Job drawing, mm, ordinate dimensions from the low corner. One solid piece. A direction names the side the tool comes from. Give positions to 0.01 mm unless a question says otherwise; leave off trailing zeros. Loops run counter-clockwise (first coordinate to the right, second up) from the corner with the lowest first, then second, coordinate; pieces in that order, holes last. Notation, with made-up numbers: (31, -6) - (80, -6) arc R31 ccw to (80, 33) - close; hole circle Ø3 at (-19, 24). An arc over 180 degrees is marked (long way). Answer as CSV lines item,"result". Start each with the question number.
Item 1: Pull direction Z, two halves, no side cores. Call the marked faces 1, 2 and 3: pulls with the +Z half, pulls with the -Z half, needs draft (parallel to the pull), parting line crosses it, or undercut.
Item 2: Saw through at B-B on y = 6.5. Give the cut face in (x, z).
Item 3: Saw through at D-D on z = 29.5. Give the cut face in (x, y), plus the area to 3 significant figures.
Item 4: Drill centre lines: L1, parallel to Z at x = 60, y = 3.9; L2, parallel to X at y = 4, z = 50; L3, parallel to Z at x = 23, y = 5.5. Where is each one in solid material? Low to high. Write a range as from..to.
Item 5: Saw through at A-A on x = 60. Give the cut face in (y, z), plus the area to 3 significant figures.
Item 6: Saw through at C-C on z = 15. Give the cut face in (x, y).
Item 7: Tool access for the marked faces 4, 5 and 6: list every direction of +Z, -Z, +X, -X, +Y, -Y with a clear straight run to the whole face (end or side of a thin tool).
Item 8: Pin check, flat tips, straight feed: pin 1 (19.5 mm diameter, centred on x = 43.5, z = 41, fed in from +Y); pin 2 (8 mm diameter, centred on x = 60, z = 15, fed in from -Y); pin 3 (3 mm diameter, centred on y = 26, z = 46, fed in from +X). Stop position of each tip, or through.
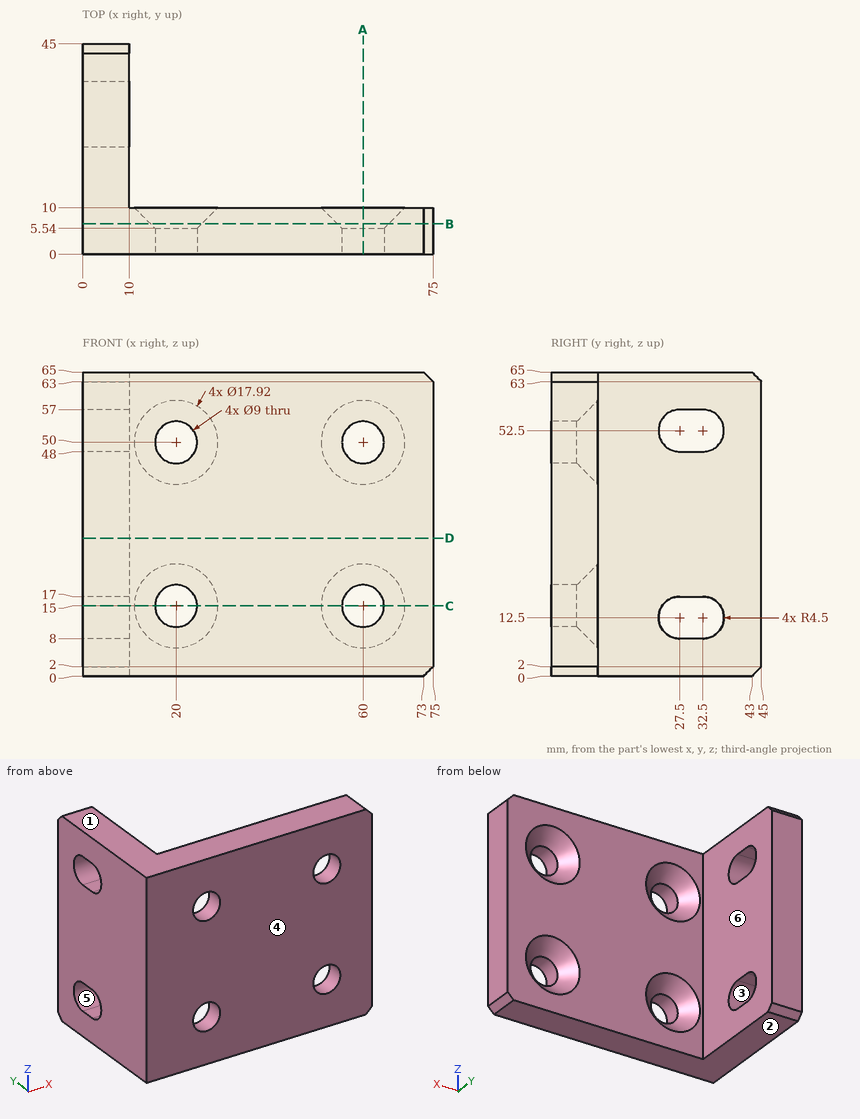
Responses:
1,face 1,"pulls with the +Z half"
1,face 2,"pulls with the -Z half"
1,face 3,"undercut"
2,outline,"(0, 0) - (73, 0) - (75, 2) - (75, 63) - (73, 65) - (0, 65) - close; hole circle Ø10.92 at (20, 15); hole circle Ø10.92 at (20, 50); hole circle Ø10.92 at (60, 15); hole circle Ø10.92 at (60, 50)"
3,outline,"(0, 0) - (75, 0) - (75, 10) - (10, 10) - (10, 45) - (0, 45) - close"
3,area,"1,100 mm2"
4,L1,"0..10.5, 19.5..45.5, 54.5..65"
4,L2,"0..15.5, 24.5..55.5, 64.5..75"
4,L3,"0..11.65, 18.35..46.65, 53.35..65"
5,outline,"(0, 0) - (10, 0) - (10, 6.04) - (5.54, 10.5) - (0, 10.5) - close; (0, 19.5) - (5.54, 19.5) - (10, 23.96) - (10, 41.04) - (5.54, 45.5) - (0, 45.5) - close; (0, 54.5) - (5.54, 54.5) - (10, 58.96) - (10, 65) - (0, 65) - close"
5,area,"430 mm2"
6,outline,"(0, 0) - (15.5, 0) - (15.5, 5.54) - (11.04, 10) - (10, 10) - (10, 23.76) - (0, 23.76) - close; (0, 36.24) - (10, 36.24) - (10, 45) - (0, 45) - close; (24.5, 0) - (55.5, 0) - (55.5, 5.54) - (51.04, 10) - (28.96, 10) - (24.5, 5.54) - close; (64.5, 0) - (75, 0) - (75, 10) - (68.96, 10) - (64.5, 5.54) - close"
7,face 4,"+Z, -Z, +X, -X, -Y"
7,face 5,"+X, -X"
7,face 6,"+Z, -Z, +X, +Y"
8,pin 1,"y = 10"
8,pin 2,"through"
8,pin 3,"x = 10"
